```python
from build123d import *

# Parameters (mm, degrees)
SKETCH1_W                                           = 420
SKETCH1_H                                           = 22
BOSS_EXTRUDE1_DEPTH                                 = 27
M5_TAPPED_HOLE1_D                                   = 4.2
M5_TAPPED_HOLE1_DEPTH                               = 12.4
M5_TAPPED_HOLE1_TIP                                 = 1.2618073
CBORE_FOR_M5_HEX_SOCKET_HEAD_CAP_SCREW1_D           = 5.5
CBORE_FOR_M5_HEX_SOCKET_HEAD_CAP_SCREW1_CBORE_D     = 10
CBORE_FOR_M5_HEX_SOCKET_HEAD_CAP_SCREW1_CBORE_DEPTH = 17


with BuildPart() as part:
    # Sketch1 → Boss-Extrude1 (new body)
    with BuildSketch(Plane.XY):
        Rectangle(SKETCH1_W, SKETCH1_H)
    extrude(amount=BOSS_EXTRUDE1_DEPTH)

    # M5 Tapped Hole1
    with Locations(Plane.XY.offset(27)):
        with Locations((-180, 1), (-120, 1), (-60, 1), (0, 1), (60, 1), (120, 1), (180, 1)):
            Hole(M5_TAPPED_HOLE1_D / 2, depth=M5_TAPPED_HOLE1_DEPTH)
            with Locations((0, 0, -(M5_TAPPED_HOLE1_DEPTH + M5_TAPPED_HOLE1_TIP / 2))):  # 118° drill point
                Cone(0, M5_TAPPED_HOLE1_D / 2, M5_TAPPED_HOLE1_TIP, mode=Mode.SUBTRACT)

    # CBORE for M5 Hex Socket Head Cap Screw1 (through all)
    with Locations(Plane.XY.offset(27)):
        with Locations((-200, 0), (-80, 0), (80, 0), (200, 0)):
            CounterBoreHole(CBORE_FOR_M5_HEX_SOCKET_HEAD_CAP_SCREW1_D / 2, CBORE_FOR_M5_HEX_SOCKET_HEAD_CAP_SCREW1_CBORE_D / 2, CBORE_FOR_M5_HEX_SOCKET_HEAD_CAP_SCREW1_CBORE_DEPTH)


solid = part.part
```
Part model, mm, in its own coordinate system. A direction names the side the tool comes from. Coordinates: 2 decimals unless noted, no trailing zeros. Write item = value, one per line. Start each with the question number.
Item 1: 3-axis set-ups, long thin cutter, end or side, ignore diameter. For faces 1 (the flat face through (-77.8, -2.2, 10)), 2 (the flat face through (-3, 0, 0)): which of +Z, -Z, +X, -X, +Y, -Y reach the whole face in a straight line?
Item 2: Flat gauge pins, fed straight in: pin 1 Ø9 at (x, y) = (80, 0) entering from +Z; pin 2 Ø2.5 at (x, y) = (-180, 1) entering from +Z; pin 3 Ø4.5 at (x, y) = (-200, 0) entering from -Z. Where does each tip first touch, or does it go through?
Item 3: Wall check: L1, parallel to Y at x = 60, z = 19.5; L2, parallel to X at y = 4.25, z = 23; L3, parallel to X at y = -2.25, z = 24.25. Give the ranges that are in metal, low to high. Write a range as from..to.
Item 4: Mould opens along X. For faces 3 (the flat face through (-210, 0, 13)), 4 (the flat face through (-3, 0, 27)), 5 (the flat face through (210, 0, 13)), 6 (the cylindrical face through (84.619, -1.915, 18.619)) say: released by +X, released by -X, zero draft, split by the parting line, or undercut.
The answers:
q1.face_1 = +Z
q1.face_2 = -Z, +X, -X, +Y, -Y
q2.pin_1 = 10
q2.pin_2 = 14.09
q2.pin_3 = through
q3.L1 = -11..-1.1, 3.1..11
q3.L2 = -210..-202.63, -197.37..-82.63, -77.37..77.37, 82.63..197.37, 202.63..210
q3.L3 = -210..-204.47, -195.53..-84.47, -75.53..75.53, 84.47..195.53, 204.47..210
q4.face_3 = released by -X
q4.face_4 = zero draft
q4.face_5 = released by +X
q4.face_6 = undercut
